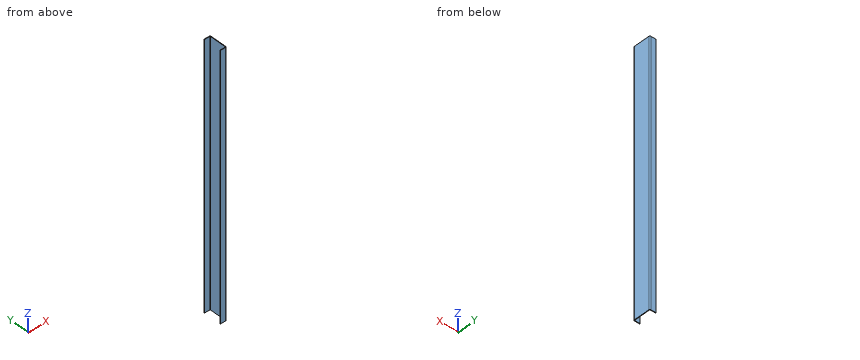
```python
from build123d import *

# Parameters (mm, degrees)
BOSS_EXTRUDE1_DEPTH = 1062


with BuildPart() as part:
    # Sketch1 → Boss-Extrude1 (new, symmetric)
    with BuildSketch(Plane.XY):
        with BuildLine():
            Line((-50, -72.5), (-8, -72.5))
            ThreePointArc((-8, -72.5), (-2.343145751, -70.156854249), (0, -64.5))
            Line((0, -64.5), (0, 64.5))
            ThreePointArc((0, 64.5), (-2.343145751, 70.156854249), (-8, 72.5))
            Line((-8, 72.5), (-50, 72.5))
            Line((-50, 72.5), (-50, 68.5))
            Line((-50, 68.5), (-8, 68.5))
            ThreePointArc((-8, 68.5), (-5.171572875, 67.328427125), (-4, 64.5))
            Line((-4, 64.5), (-4, -64.5))
            ThreePointArc((-4, -64.5), (-5.171572875, -67.328427125), (-8, -68.5))
            Line((-8, -68.5), (-50, -68.5))
            Line((-50, -68.5), (-50, -72.5))
        make_face()
    extrude(amount=BOSS_EXTRUDE1_DEPTH, both=True)


solid = part.part
```
The listing builds one solid part. Answer for the finished solid, in the listing's coordinates (mm). Round coordinates to 2 decimals unless told otherwise and drop trailing zeros. Write each loop counter-clockwise with the first axis right and the second up, starting at its lowest first coordinate (ties: lowest second). Pieces come first, ordered by that corner, then holes. Notation, with made-up numbers: (-29, 24) -> (-21, 24) arc R32 cw to (-21, 58) -> close; hole circle Ø7 at (22.5, 64.25). An arc over 180 degrees is marked (long way). Use CSV: the item, a comma, the result in double quotes. Start each with the question number.
(1) Section C-C on y = -29 is taken. Give the vertices of the cut face in (x, z), then the cut area to 3 significant figures.
(2) This flat-tipped pin is pushed along its axis until it touches: pin 1 (12 mm diameter, centred on y = -56, z = 118.5, fed in from -X). Where does it stop, or does it pass through?
(3) Section B-B on z = 34 is taken. Give the vertices of the cut face in (x, y), then the cut area to 3 significant figures.
(4) Section A-A on x = -38 is taken. Give the vertices of the cut face in (y, z).
(5) Consider L1, parallel to Y at x = -27, z = -860; L2, parallel to X at y = 54.5, z = 662.5. Determine where each line is inside the solid, lowest interval first. Write a range as from..to.
A:
1,outline,"(-4, -1062) -> (0, -1062) -> (0, 1062) -> (-4, 1062) -> close"
1,area,"8,500 mm²"
2,pin 1,"stops at x = -4"
3,outline,"(-50, -72.5) -> (-8, -72.5) arc R8 ccw to (0, -64.5) -> (0, 64.5) arc R8 ccw to (-8, 72.5) -> (-50, 72.5) -> (-50, 68.5) -> (-8, 68.5) arc R4 cw to (-4, 64.5) -> (-4, -64.5) arc R4 cw to (-8, -68.5) -> (-50, -68.5) -> close"
3,area,"927 mm²"
4,outline,"(-72.5, -1062) -> (-68.5, -1062) -> (-68.5, 1062) -> (-72.5, 1062) -> close; (68.5, -1062) -> (72.5, -1062) -> (72.5, 1062) -> (68.5, 1062) -> close"
5,L1,"y = -72.5..-68.5, 68.5..72.5"
5,L2,"x = -4..0"
